Check sheet for the drawn part. Datum: minimum x, y, z corner. Units: mm. Coordinates: 2 decimals unless noted, no trailing zeros. Write each loop counter-clockwise with the first axis right and the second up, starting at its lowest first coordinate (ties: lowest second). Pieces come first, ordered by that corner, then holes. Notation, with made-up numbers: (32, 51) - (39, 51) arc R27 ccw to (39, 70) - close; hole circle Ø6 at (-16, 15). An arc over 180 degrees is marked (long way). Write each question's results on one line, items separated by ' | '.
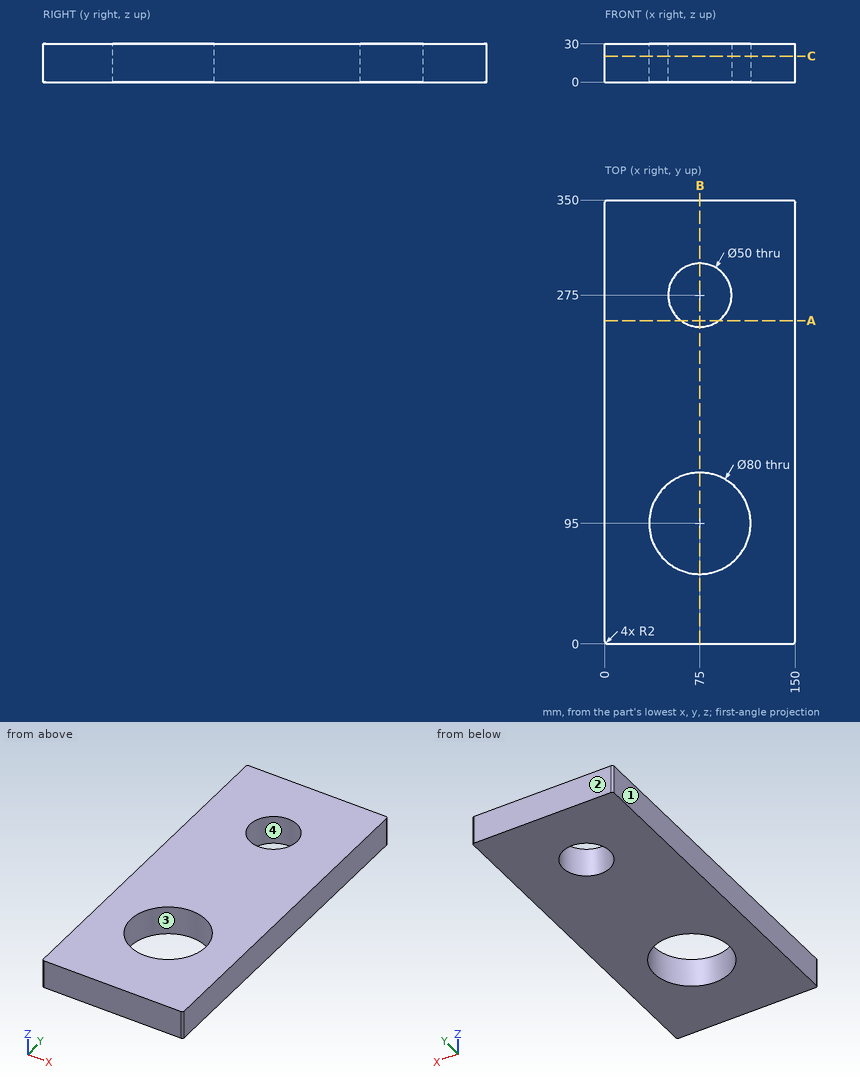
1. Sectioned sample at B-B (x = 75). Record the cut outline in (y, z), then the cut area to 3 significant figures.
Values follow:
outline: (0, 0) - (55, 0) - (55, 30) - (0, 30) - close; (135, 0) - (250, 0) - (250, 30) - (135, 30) - close; (300, 0) - (350, 0) - (350, 30) - (300, 30) - close | area: 6,600 mm^2
2. Material ranges on L1, parallel to Y at x = 75, z = 9; L2, parallel to Y at x = 77.5, z = 26.25; L3, parallel to X at y = 121.5, z = 23.5, recorded low to high. Write a range as [from, to].
Values follow:
L1: y = [0, 55], [135, 250], [300, 350] | L2: y = [0, 55.08], [134.92, 250.13], [299.87, 350] | L3: x = [0, 45.04], [104.96, 150]
3. Sectioned sample at C-C (z = 20.5). Record the cut outline in (x, y), then the cut area to 3 significant figures.
Values follow:
outline: (0, 2) arc R2 ccw to (2, 0) - (148, 0) arc R2 ccw to (150, 2) - (150, 348) arc R2 ccw to (148, 350) - (2, 350) arc R2 ccw to (0, 348) - close; hole circle Ø80 at (75, 95); hole circle Ø50 at (75, 275) | area: 45,500 mm^2
4. Sectioned sample at A-A (y = 255). Record the cut outline in (x, z), then the cut area to 3 significant figures.
Values follow:
outline: (0, 0) - (60, 0) - (60, 30) - (0, 30) - close; (90, 0) - (150, 0) - (150, 30) - (90, 30) - close | area: 3,600 mm^2
5. Draft check along Y on the marked faces 1, 2, 3 and 4. Enter one of: pulls with the +Y half, pulls with the -Y half, needs draft (parallel to the pull), parting line crosses it, or undercut.
Values follow:
face 1: needs draft | face 2: pulls with the +Y half | face 3: undercut | face 4: undercut
